from build123d import *

# Parameters (mm, degrees)
SKETCH_1_W                  = 50
SKETCH_1_H                  = 290
EXTRUDE_1_DEPTH             = 20
HOLE_WIZARD_11_0_11_1_D     = 11
HOLE_WIZARD_11_0_11_1_DEPTH = 36
HOLE_WIZARD_11_0_11_1_TIP   = 3.304733405


with BuildPart() as part:
    # 草图1 → 凸台-拉伸1 (new body)
    with BuildSketch(Plane.XY):
        Rectangle(SKETCH_1_W, SKETCH_1_H)
    extrude(amount=EXTRUDE_1_DEPTH)

    # Ø11.0 (11) 直径孔1
    with Locations(Plane.XY.offset(20)):
        with Locations((-5, 125), (-5, 50), (-5, -50), (-5, -125)):
            Hole(HOLE_WIZARD_11_0_11_1_D / 2, depth=HOLE_WIZARD_11_0_11_1_DEPTH)
            with Locations((0, 0, -(HOLE_WIZARD_11_0_11_1_DEPTH + HOLE_WIZARD_11_0_11_1_TIP / 2))):  # 118° drill point
                Cone(0, HOLE_WIZARD_11_0_11_1_D / 2, HOLE_WIZARD_11_0_11_1_TIP, mode=Mode.SUBTRACT)


solid = part.part
Design review of the part built by this model. Coordinates are the model's own, in mm. Give positions to 0.01 mm unless a question says otherwise; leave off trailing zeros. Loops run counter-clockwise (first coordinate to the right, second up) from the corner with the lowest first, then second, coordinate; pieces in that order, holes last. Notation, with made-up numbers: M 46,30.5 L 57,30.5 A19 ccw 57,48.5 Z; hole C 85.5,59.5 d1. An arc over 180 degrees is marked long. One line per question, with ' | ' between items. Start each with the question number.
1. To check wall thickness, follow L1, parallel to Y at x = -5, z = 6; L2, parallel to Y at x = -8, z = 4.75. State the ranges of each line that lie inside material, in increasing order.
2. Add section A-A (y = -125). Write out the cut boundary in (x, z).
3. Insertion check: P1, Ø17.5, axis at x = -5, y = 50, coming from the -Z side; P2, Ø10, axis at x = -5, y = -125, coming from the +Z side. Each pin has a flat end and moves straight along its axis. Give the tip position at first contact, or say it passes through.
4. Add section B-B (z = 4). Write out the cut boundary in (x, y), plus the area to 3 significant figures.
5. The part is to be moulded in two halves that separate along X. For faces 1 (the face through (-4.284, -119.547, 9.86)), 2 (the face through (0, 2, 20)), 3 (the face through (-4.284, 55.453, 9.86)), 4 (the face through (25, -2, 10)), say which applies: released by +X, released by -X, zero draft, split by the parting line, or undercut.
Worked out:
1) L1: y = -145 to -130.5, -119.5 to -55.5, -44.5 to 44.5, 55.5 to 119.5, 130.5 to 145 | L2: y = -145 to -129.61, -120.39 to -54.61, -45.39 to 45.39, 54.61 to 120.39, 129.61 to 145
2) outline: M -25,0 L -10.5,0 L -10.5,20 L -25,20 Z; M 0.5,0 L 25,0 L 25,20 L 0.5,20 Z
3) P1: stops at z = 0 | P2: passes through
4) outline: M -25,-145 L 25,-145 L 25,145 L -25,145 Z; hole C -5,-125 d11; hole C -5,-50 d11; hole C -5,50 d11; hole C -5,125 d11 | area: 14,100 mm²
5) face 1: undercut | face 2: zero draft | face 3: undercut | face 4: released by +X
